Geometry: final body of the model. Coordinates: model frame, mm. Give positions to 0.01 mm unless a question says otherwise; leave off trailing zeros. Write each loop counter-clockwise with the first axis right and the second up, starting at its lowest first coordinate (ties: lowest second). Pieces come first, ordered by that corner, then holes. Notation, with made-up numbers: M 80.5,50 L 101.5,50 A21 cw 101.5,59 Z; hole C 47.5,50.25 d3. An arc over 180 degrees is marked long. Use one line per item in the form item = value. Start each with the question number.
Item 1: Material intervals for line 1 along Y through (x, z) = (22.25, -7); line 2 along Y through (x, z) = (4.75, -127.5), sorted ascending. Write a range as from..to.
Item 2: Contact query for flat-ended pins moving along their axis: P1, Ø10, axis at y = 25.5, z = -119.5, coming from the +X side; P2, Ø10, axis at x = 11, y = 17.5, coming from the +Z side; P3, Ø5, axis at y = 6, z = -151, coming from the +X side. Output: stop coordinate, or through.
Item 3: Section query B-B on y = 16. Return loops of the section in (x, z).
Item 4: Section query A-A on z = 124. Return loops of the section in (x, y), then the cut area to 3 significant figures.
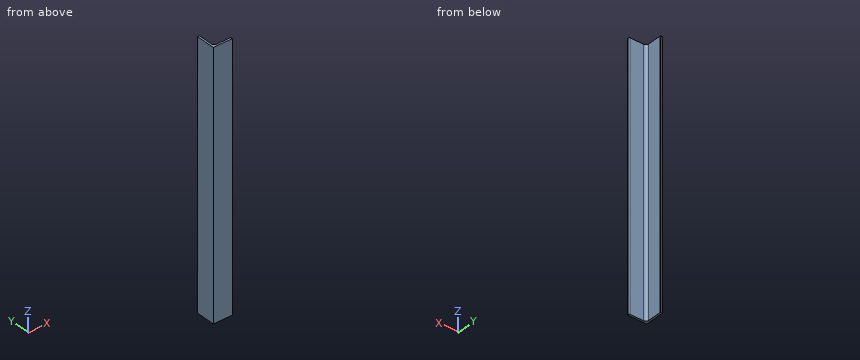
from build123d import *

# Parameters (mm, degrees)
BOSS_EXTRUDE1_DEPTH = 203.8


with BuildPart() as part:
    # Sketch1 → Boss-Extrude1 (new, symmetric)
    with BuildSketch(Plane.XY):
        with BuildLine():
            Line((0, 0), (0, 30))
            Line((0, 30), (2, 30))
            ThreePointArc((2, 30), (2.707106781, 29.707106781), (3, 29))
            Line((3, 29), (3, 7.5))
            ThreePointArc((3, 7.5), (4.318019485, 4.318019485), (7.5, 3))
            Line((7.5, 3), (29, 3))
            ThreePointArc((29, 3), (29.707106781, 2.707106781), (30, 2))
            Line((30, 2), (30, 0))
            Line((30, 0), (0, 0))
        make_face()
    extrude(amount=BOSS_EXTRUDE1_DEPTH, both=True)


solid = part.part
Answer sheet:
q1.line_1 = 0..3
q1.line_2 = 0..3.94
q2.P1 = 3
q2.P2 = through
q2.P3 = 5.44
q3.outline = M 0,-203.8 L 3,-203.8 L 3,203.8 L 0,203.8 Z
q4.outline = M 0,0 L 30,0 L 30,2 A1 ccw 29,3 L 7.5,3 A4.5 cw 3,7.5 L 3,29 A1 ccw 2,30 L 0,30 Z
q4.area = 175 mm2
